from build123d import *

# Parameters (mm, degrees)
BOSS_EXTRUDE1_DEPTH = 234.95
SKETCH2_W           = 19.05
SKETCH2_H           = 17.55
CUT_EXTRUDE1_DEPTH  = 238.849674164
CUT_EXTRUDE2_DEPTH  = 238.849674164


with BuildPart() as part:
    # Sketch1 → Boss-Extrude1 (new body)
    with BuildSketch(Plane.XY):
        with BuildLine():
            Line((30.25, 3.1), (30.25, 19.05))
            Line((30.25, 19.05), (31.75, 19.05))
            Line((31.75, 19.05), (31.75, 3.2))
            ThreePointArc((31.75, 3.2), (30.8127417, 0.9372583), (28.55, 0))
            Line((28.55, 0), (3.2, 0))
            ThreePointArc((3.2, 0), (0.9372583, 0.9372583), (0, 3.2))
            Line((0, 3.2), (0, 19.05))
            Line((0, 19.05), (1.5, 19.05))
            Line((1.5, 19.05), (1.5, 3.1))
            ThreePointArc((1.5, 3.1), (1.96862915, 1.96862915), (3.1, 1.5))
            Line((3.1, 1.5), (28.65, 1.5))
            ThreePointArc((28.65, 1.5), (29.78137085, 1.96862915), (30.25, 3.1))
        make_face()
    extrude(amount=BOSS_EXTRUDE1_DEPTH)

    # Sketch2 → Cut-Extrude1 (cut, through all)
    with BuildSketch(Plane(origin=(0, 0, 0), x_dir=(0, 0, -1), z_dir=(1, 0, 0))):
        with Locations((-9.525, 10.275)):
            Rectangle(SKETCH2_W, SKETCH2_H)
        with Locations((-225.425, 10.275)):
            Rectangle(SKETCH2_W, SKETCH2_H)
    extrude(amount=CUT_EXTRUDE1_DEPTH, mode=Mode.SUBTRACT)

    # Sketch3 → Cut-Extrude2 (cut, through all)
    with BuildSketch(Plane(origin=(0, 0, 0), x_dir=(1, 0, 0), z_dir=(0, 1, 0))):
        Polygon((22.821846385, -57.15), (8.928153615, -57.15), (8.928153615, -31.75), (9.428153615, -31.75), (9.428153615, -56.65), (22.321846385, -56.65), (22.321846385, -31.75), (22.821846385, -31.75), align=None)
    extrude(amount=CUT_EXTRUDE2_DEPTH, mode=Mode.SUBTRACT)


solid = part.part
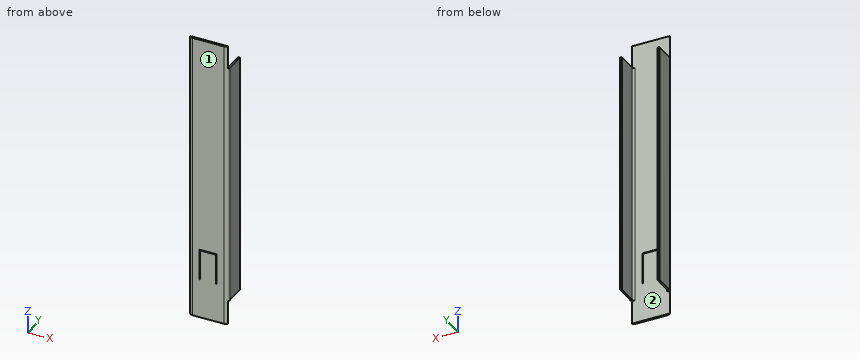
The model under review builds one solid part; all positions refer to its coordinate system, in mm. Face numbers are marked on the shaded views. Coordinates: 2 decimals unless noted, no trailing zeros. Loops run counter-clockwise (first coordinate to the right, second up) from the corner with the lowest first, then second, coordinate; pieces in that order, holes last. Notation, with made-up numbers: M 40.25,29.5 L 89.25,29.5 A28 ccw 89.25,63.5 Z; hole C 41,77 d5. An arc over 180 degrees is marked long. Put each result on its own line as item: value. Start each with the question number.
Q1. The part is to be moulded in two halves that separate along X. For the marked faces 1 and 2, say which applies: +X half, -X half, draft (parallel to the pull), parting line (faces both ways), or undercut.
Q2. Wall thickness on line 1 (X direction, y = 6.75, z = 140.5); line 2 (X direction, y = 2.75, z = 43); line 3 (Z direction, x = 11, y = 1.25): over which ranges is each line inside the solid? List them lowest first.
Q3. Clearance check with flat-ended pins moving along their axes: pin 1 (0.8 mm diameter, centred on y = 1, z = 49, fed in from +X); pin 2 (0.9 mm diameter, centred on x = 1.5, y = 14, fed in from +Z); pin 3 (0.8 mm diameter, centred on y = 1, z = 43.5, fed in from -X). State where each tip first meets the part, or that it passes through.
Q4. Add section B-B (y = 12.5). Write out the cut boundary in (x, z), and give its area (3 significant figures).
Q5. Add section A-A (x = 13.5). Write out the cut boundary in (y, z).
Q6. Add section C-C (z = 26). Write out the cut boundary in (x, y), and give its area (3 significant figures).
Answers:
1. face 1: draft
1. face 2: undercut
2. line 1: x = 0 to 1.5, 30.25 to 31.75
2. line 2: x = 0.03 to 1.54, 30.21 to 31.72
2. line 3: z = 0 to 56.65, 57.15 to 234.95
3. pin 1: stops at x = 31.2
3. pin 2: stops at z = 215.9
3. pin 3: stops at x = 0.55
4. outline: M 0,19.05 L 1.5,19.05 L 1.5,215.9 L 0,215.9 Z; M 30.25,19.05 L 31.75,19.05 L 31.75,215.9 L 30.25,215.9 Z
4. area: 591 mm^2
5. outline: M 0,0 L 1.5,0 L 1.5,56.65 L 0,56.65 Z; M 0,57.15 L 1.5,57.15 L 1.5,234.95 L 0,234.95 Z
6. outline: M 0,3.2 A3.2 ccw 3.2,0 L 28.55,0 A3.2 ccw 31.75,3.2 L 31.75,19.05 L 30.25,19.05 L 30.25,3.1 A1.6 cw 28.65,1.5 L 3.1,1.5 A1.6 cw 1.5,3.1 L 1.5,19.05 L 0,19.05 Z
6. area: 97.0 mm^2
